Design review of the part built by this model. Coordinates are the model's own, in mm. A direction names the side the tool comes from. Coordinates: 2 decimals unless noted, no trailing zeros. Write each loop counter-clockwise with the first axis right and the second up, starting at its lowest first coordinate (ties: lowest second). Pieces come first, ordered by that corner, then holes. Notation, with made-up numbers: (-6, -17) -> (27, -17) arc R9 ccw to (27, -4) -> close; hole circle Ø11 at (71.25, 50). An arc over 180 degrees is marked (long way). One line per question, with ' | ' between items. Start each with the question number.
Q1. Add section C-C on z = 1.3. State the section outline as (x, y) points.
Q2. Add section A-A on x = 0. State the section outline as (y, z) points.
Q3. Add section B-B on y = 0. State the section outline as (x, z) points.
Q4. Draft analysis for pull direction X (two halves, no side actions). For faces 4 (the conical face through (0.12, 5.81, 0.11)), 5 (the flat face through (-5, 0, 1.5)), 6 (the cylindrical face through (3.34, 1.05, 2.22)), state which applies: pulls with the +X half, pulls with the -X half, needs draft (parallel to the pull), parting line crosses it, or undercut.
Q5. For P1, Ø0.5, axis at x = 4.5, z = 1, coming from the -Y side; P2, Ø1, axis at x = 1.5, z = 2, coming from the -Y side; P3, Ø1.2, axis at x = -4.5, z = 1, coming from the -Y side, all flat-tipped, find the tip position at first contact; note any pin that passes through.
Q6. Wall thickness on probe 1 along Y at (x, z) = (0, 1.9); probe 2 along Z at (x, y) = (-4.75, -2.5): over which ranges is each line inside the solid? List them lowest first.
Q7. For faces 1 (the cylindrical face through (5, 1.6, 4.5)), 2 (the flat face through (0, 4, 0)), 3 (the flat face through (5, 0, 1.5)), list the 3-axis set-ups (+Z, -Z, +X, -X, +Y, -Y) from which the entire face can be reached by the end or side of a thin tool; tool diameter is ignored.
from build123d import *

# Parameters (mm, degrees)
SKETCH_1_R          = 6
SKETCH_1_R_2        = 3.5
EXTRUDE_1_DEPTH     = 5
CHAMFER_1_SIZE      = 0.5
SKETCH_2_W          = 16.841160442
SKETCH_2_H          = 1
CUT_EXTRUDE_1_DEPTH = 1.5
CUT_EXTRUDE_START   = -1
SKETCH_3_R          = 6
SKETCH_3_R_2        = 5.25
CUT_EXTRUDE_2_DEPTH = 1
CHAMFER_2_SIZE      = 0.3


with BuildPart() as part:
    # 草图1 → 凸台-拉伸1 (new body)
    with BuildSketch(Plane.XY):
        Circle(SKETCH_1_R)
        Circle(SKETCH_1_R_2, mode=Mode.SUBTRACT)
    extrude(amount=EXTRUDE_1_DEPTH)

    # 倒角1
    chamfer_1_edges = [part.edges().sort_by_distance(p)[0] for p in [
        (-3.5, 0, 5),
    ]]
    chamfer(chamfer_1_edges, length=CHAMFER_1_SIZE)

    # 草图2 → 切除-拉伸1 (cut)
    with BuildSketch(Plane(origin=(0, 0, 0), x_dir=(-1, 0, 0), z_dir=(0, 0, -1))):
        with Locations((-0.328074554, 0)):
            Rectangle(SKETCH_2_W, SKETCH_2_H)
    extrude(amount=-CUT_EXTRUDE_1_DEPTH, mode=Mode.SUBTRACT)

    # 草图3 → 切除-拉伸2 (cut)
    with BuildSketch(Plane.XY.offset(5).offset(CUT_EXTRUDE_START)):
        with Locations(Location((0, 0, 0), (0, 0, 175.219808153))):
            Circle(SKETCH_3_R)
        Circle(SKETCH_3_R_2, mode=Mode.SUBTRACT)
    extrude(amount=CUT_EXTRUDE_2_DEPTH, mode=Mode.SUBTRACT)

    # 倒角2
    chamfer_2_edges = [part.edges().sort_by_distance(p)[0] for p in [
        (0, -6, 0),
        (0, 6, 0),
        (-6, 0, 4),
    ]]
    chamfer(chamfer_2_edges, length=CHAMFER_2_SIZE)


solid = part.part
Output values:
1) outline: (-5.98, -0.5) arc R6 ccw to (5.98, -0.5) -> (3.46, -0.5) arc R3.5 cw to (-3.46, -0.5) -> close; (-5.98, 0.5) -> (-3.46, 0.5) arc R3.5 cw to (3.46, 0.5) -> (5.98, 0.5) arc R6 ccw to start
2) outline: (-6, 0.3) -> (-5.7, 0) -> (-3.5, 0) -> (-3.5, 4.5) -> (-4, 5) -> (-5.25, 5) -> (-5.25, 4) -> (-5.7, 4) -> (-6, 3.7) -> close; (3.5, 0) -> (5.7, 0) -> (6, 0.3) -> (6, 3.7) -> (5.7, 4) -> (5.25, 4) -> (5.25, 5) -> (4, 5) -> (3.5, 4.5) -> close
3) outline: (-6, 1.5) -> (-3.5, 1.5) -> (-3.5, 4.5) -> (-4, 5) -> (-5.25, 5) -> (-5.25, 4) -> (-5.7, 4) -> (-6, 3.7) -> close; (3.5, 1.5) -> (6, 1.5) -> (6, 3.7) -> (5.7, 4) -> (5.25, 4) -> (5.25, 5) -> (4, 5) -> (3.5, 4.5) -> close
4) face 4: parting line crosses it | face 5: needs draft | face 6: undercut
5) P1: stops at y = -4.24 | P2: stops at y = -5.92 | P3: stops at y = -4.56
6) probe 1: y = -6 to -3.5, 3.5 to 6 | probe 2: z = 0 to 4
7) face 1: +Z | face 2: -Z, +X, -X, +Y, -Y | face 3: -Z, +X, -X
